from build123d import *

# Parameters (mm, degrees)
FORKED_BASE_DEPTH   = 18
UPRIGHT_BOSS_DEPTH  = 14
NOTCH_SKETCH_8X9_W  = 8
NOTCH_SKETCH_8X9_H  = 9
NOTCH_CUT_8X9_DEPTH = 93.854725243


with BuildPart() as part:
    # Base Profile Sketch → Forked Base (new body)
    with BuildSketch(Plane.XY):
        Polygon((-23, 15), (-7, 22), (7, 22), (23, 15), (23, -15), (-23, -15), align=None)
    extrude(amount=FORKED_BASE_DEPTH)

    # Upright Profile Sketch → Upright Boss (add)
    with BuildSketch(Plane(origin=(0, -15, 0), x_dir=(-1, 0, 0), z_dir=(0, -1, 0))):
        with BuildLine():
            Line((-23, -18), (-23, -44))
            Line((-23, -44), (-18, -82))
            Line((-18, -82), (-7, -82))
            Line((-7, -82), (-7, -60))
            ThreePointArc((-7, -60), (0, -53), (7, -60))
            Line((7, -60), (7, -82))
            Line((7, -82), (18, -82))
            Line((18, -82), (23, -44))
            Line((23, -44), (23, -18))
            Line((23, -18), (-23, -18))
        make_face()
    extrude(amount=-UPRIGHT_BOSS_DEPTH)

    # Notch Sketch 8x9 → Notch Cut 8x9 (cut, through all)
    with BuildSketch(Plane.XZ.offset(15)):
        with Locations((19, 4.5)):
            Rectangle(NOTCH_SKETCH_8X9_W, NOTCH_SKETCH_8X9_H)
    notch_cut_8x9 = extrude(amount=-NOTCH_CUT_8X9_DEPTH, mode=Mode.SUBTRACT)

    # Notch Mirror: Notch Cut 8x9 across plane
    add(notch_cut_8x9.mirror(Plane(origin=(0, 0, 0), x_dir=(0, 0, 1), z_dir=(1, 0, 0))), mode=Mode.SUBTRACT)


solid = part.part
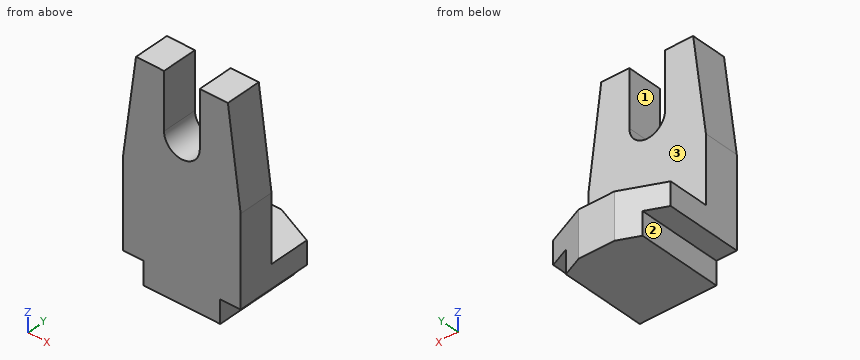
The listing builds one solid part. Answer for the finished solid, in the listing's coordinates (mm). Face numbers are marked on the shaded views. A direction names the side the tool comes from. Coordinates: 2 decimals unless noted, no trailing zeros. Order: outer loops, then holes, each group sorted by start corner. A loop starts at its lowest first (then second) coordinate and runs counter-clockwise, first axis right, second up.
Q1. Consider line 1 (Z direction, x = -8.5, y = 3.5); line 2 (Z direction, x = -16, y = 1.5); line 3 (Y direction, x = -16, z = 30). Determine where each line is inside the solid, lowest interval first.
Q2. Given P1, Ø14, axis at x = 8.5, z = 65.5, coming from the +Y side; P2, Ø8, axis at y = -7, z = 53, coming from the -X side; P3, Ø6, axis at y = 1, z = 73, coming from the +X side, each flat-ended and moving along its own axis, determine where each tip first touches the part or whether it passes through.
Q3. A cutting plane is placed at C-C, the plane x = 0. Write down the section's boundary in (y, z), and give its area (3 significant figures).
Q4. A cutting plane is placed at A-A, the plane y = -7. Write down the section's boundary in (x, z), and give its area (3 significant figures).
Q5. Which of the six approach directions +Z, -Z, +X, -X, +Y, -Y give full straight-line access (tool end or side, diameter ignored) to the marked faces 1, 2 and 3?
Q6. A cutting plane is placed at B-B, the plane z = 74. Write down the section's boundary in (x, y).
Q7. A cutting plane is placed at D-D, the plane y = 12. Write down the section's boundary in (x, z).
Answers follow:
1. line 1: z = 0 to 18
1. line 2: z = 9 to 18
1. line 3: y = -15 to -1
2. P1: stops at y = -1
2. P2: stops at x = -22.34
2. P3: stops at x = 19.48
3. outline: (-15, 0) - (22, 0) - (22, 18) - (-1, 18) - (-1, 53) - (-15, 53) - close
3. area: 1,160 mm2
4. outline: (-23, 9) - (-15, 9) - (-15, 0) - (15, 0) - (15, 9) - (23, 9) - (23, 44) - (18, 82) - (7, 82) - (7, 60) arc R7 cw to (-7, 60) - (-7, 82) - (-18, 82) - (-23, 44) - close
4. area: 3,050 mm2
5. face 1: +Z, +Y, -Y
5. face 2: -Z, -X, +Y, -Y
5. face 3: +Z, +X, -X, +Y
6. outline: (-19.05, -15) - (-7, -15) - (-7, -1) - (-19.05, -1) - close; (7, -15) - (19.05, -15) - (19.05, -1) - (7, -1) - close
7. outline: (-23, 9) - (-15, 9) - (-15, 0) - (15, 0) - (15, 9) - (23, 9) - (23, 18) - (-23, 18) - close
